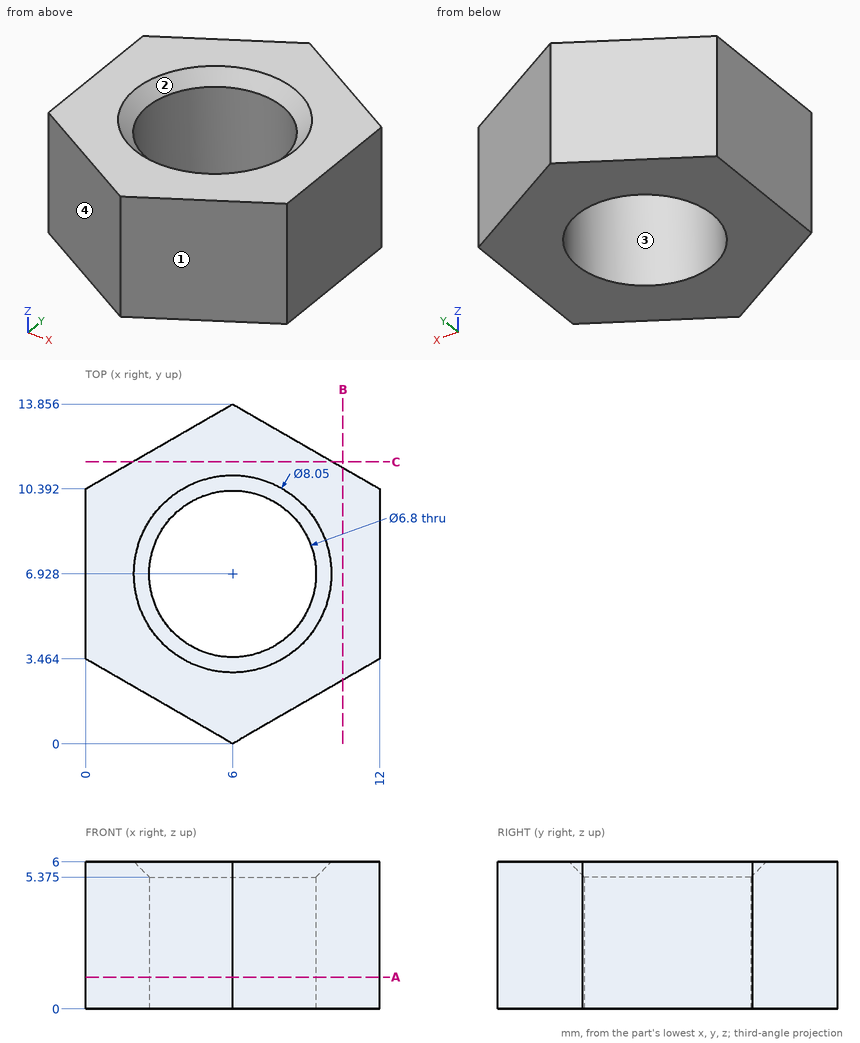
Geometry check sheet. Reference: drawing and pictorial views, mm from the part's lowest x, y, z. Coordinates: 2 decimals unless noted, no trailing zeros. Order: outer loops, then holes, each group sorted by start corner. A loop starts at its lowest first (then second) coordinate and runs counter-clockwise, first axis right, second up. Notation, with made-up numbers: M -37,16.5 L 13,16.5 A8 cw 13,20.5 Z; hole C 33,12 d2. An arc over 180 degrees is marked long. Return JSON: item names as keys, results as strings.
1) Cross-section at A-A, the plane z = 1.3. Record the boundary of the cut face in (x, y).
Answer list:
{"outline": "M 0,3.46 L 6,0 L 12,3.46 L 12,10.39 L 6,13.86 L 0,10.39 Z; hole C 6,6.93 d6.8"}
2) Release check for a two-part mould opening along X. For the marked faces 1, 2, 3 and 4 record: +X half, -X half, draft (parallel to the pull), parting line (faces both ways), or undercut.
Answer list:
{"face 1": "+X half", "face 2": "undercut", "face 3": "undercut", "face 4": "-X half"}
3) Thickness scan on L1, parallel to Y at x = 8.5, z = 4.95 (1 decimal); L2, parallel to Y at x = 3, z = 3.1 (1 decimal); L3, parallel to X at y = 9.5, z = 5.45 (1 decimal). Record the ranges inside material, lowest first. Write a range as [from, to].
Answer list:
{"L1": "[1.4, 4.6], [9.2, 12.4]", "L2": "[1.7, 5.3], [8.5, 12.1]", "L3": "[0, 3.7], [8.3, 12]"}
4) Cross-section at C-C, the plane y = 11.5. Record the boundary of the cut face in (x, z), and give its area (3 significant figures).
Answer list:
{"outline": "M 1.92,0 L 10.08,0 L 10.08,6 L 1.92,6 Z", "area": "49.0 mm2"}
5) Gauge pin test, flat end, axial feed: pin 1 (1 mm diameter, centred on y = 8.5, z = 3.5, fed in from -X). Record the tip position at first contact, or that the pin passes through.
Answer list:
{"pin 1": "x = 0"}
6) Cross-section at B-B, the plane x = 10.5. Record the boundary of the cut face in (y, z).
Answer list:
{"outline": "M 2.6,0 L 11.26,0 L 11.26,6 L 2.6,6 Z"}
